Could you check a few things on this model? Use its own coordinates, in mm. A direction names the side the tool comes from. Give positions to 0.01 mm unless a question says otherwise; leave off trailing zeros. Loops run counter-clockwise (first coordinate to the right, second up) from the corner with the lowest first, then second, coordinate; pieces in that order, holes last. Notation, with made-up numbers: (-0.75, 79) - (44.25, 79) arc R14 ccw to (44.25, 84) - close; hole circle Ø7 at (-27, 71.25). An arc over 180 degrees is marked (long way). Use CSV: the item, a comma, the result in double quotes.
from build123d import *

# Parameters (mm, degrees)
SKETCH1_W           = 29
SKETCH1_H           = 15
SKETCH1_R           = 2
SKETCH1_R_2         = 1.5
BOSS_EXTRUDE1_DEPTH = 13
SKETCH3_W           = 4.75
SKETCH3_H           = 13
SKETCH3_W_2         = 18.25
CUT_EXTRUDE1_DEPTH  = 4
SKETCH5_W           = 29
SKETCH5_H           = 4
CUT_EXTRUDE2_DEPTH  = 27
SKETCH6_W           = 1.5
SKETCH6_H           = 7
CUT_EXTRUDE3_DEPTH  = 27
SKETCH7_W           = 27.5
SKETCH7_H           = 7
CUT_EXTRUDE4_DEPTH  = 7
CHAMFER1_SIZE       = 6
CHAMFER1_SIZE2      = 4
SKETCH8_W           = 6.5
SKETCH8_H           = 0.5
CUT_EXTRUDE5_DEPTH  = 9
SKETCH9_R           = 1.25
CUT_EXTRUDE6_DEPTH  = 3.25
SKETCH12_W          = 3
SKETCH12_H          = 7
CUT_EXTRUDE8_DEPTH  = 8
SKETCH13_R          = 1.5
CUT_EXTRUDE9_DEPTH  = 8
CHAMFER3_SIZE       = 1
SKETCH17_W          = 1.5
SKETCH17_H          = 7
CUT_EXTRUDE11_DEPTH = 9
CHAMFER4_SIZE       = 2
M2_TAPPED_HOLE1_D   = 1.6


with BuildPart() as part:
    # Sketch1 → Boss-Extrude1 (new body)
    with BuildSketch(Plane.XY):
        Rectangle(SKETCH1_W, SKETCH1_H)
        with Locations(Location((6.75, 0, 0), (0, 0, 180))):
            Circle(SKETCH1_R, mode=Mode.SUBTRACT)
        with Locations(Location((-4.75, 0, 0), (0, 0, 180))):
            Circle(SKETCH1_R_2, mode=Mode.SUBTRACT)
    extrude(amount=BOSS_EXTRUDE1_DEPTH)

    # Sketch3 → Cut-Extrude1 (cut)
    with BuildSketch(Plane.XZ.offset(7.5)):
        with Locations((12.125, 6.5)):
            Rectangle(SKETCH3_W, SKETCH3_H)
        with Locations((-5.375, 6.5)):
            Rectangle(SKETCH3_W_2, SKETCH3_H)
    extrude(amount=-CUT_EXTRUDE1_DEPTH, mode=Mode.SUBTRACT)

    # Sketch5 → Cut-Extrude2 (cut)
    with BuildSketch(Plane(origin=(0, 0, 0), x_dir=(-1, 0, 0), z_dir=(0, 0, -1))):
        with Locations((0, 5.5)):
            Rectangle(SKETCH5_W, SKETCH5_H)
    extrude(amount=-CUT_EXTRUDE2_DEPTH, mode=Mode.SUBTRACT)

    # Sketch6 → Cut-Extrude3 (cut)
    with BuildSketch(Plane(origin=(0, 0, 0), x_dir=(-1, 0, 0), z_dir=(0, 0, -1))):
        with Locations((13.75, 0)):
            Rectangle(SKETCH6_W, SKETCH6_H)
    extrude(amount=-CUT_EXTRUDE3_DEPTH, mode=Mode.SUBTRACT)

    # Sketch7 → Cut-Extrude4 (cut)
    with BuildSketch(Plane(origin=(0, 0, 0), x_dir=(-1, 0, 0), z_dir=(0, 0, -1))):
        with Locations((-0.75, 0)):
            Rectangle(SKETCH7_W, SKETCH7_H)
    extrude(amount=-CUT_EXTRUDE4_DEPTH, mode=Mode.SUBTRACT)

    # Chamfer1
    chamfer1_edges = [part.edges().sort_by_distance(p)[0] for p in [
        (6.75, -7.5, 13),
    ]]
    chamfer1_side = [part.faces().sort_by_distance(p)[0] for p in [
        (6.75, -7.5, 6.5),
    ]]
    chamfer(chamfer1_edges, length=CHAMFER1_SIZE, length2=CHAMFER1_SIZE2, reference=chamfer1_side[0])

    # Sketch8 → Cut-Extrude5 (cut)
    with BuildSketch(Plane(origin=(0, 0, 7), x_dir=(-1, 0, 0), z_dir=(0, 0, -1))):
        Polygon((-1.75, -3.5), (-1.75, -0.25), (3.75, -0.25), (3.75, 0.25), (-2.25, 0.25), (-2.25, -3.5), align=None)
        with Locations((-11.25, 0)):
            Rectangle(SKETCH8_W, SKETCH8_H)
    extrude(amount=-CUT_EXTRUDE5_DEPTH, mode=Mode.SUBTRACT)

    # Sketch9 → Cut-Extrude6 (cut)
    with BuildSketch(Plane.XZ.offset(3.5)):
        with Locations((12.3, 10)):
            Circle(SKETCH9_R)
        with Locations((-0.7, 10)):
            Circle(SKETCH9_R)
    extrude(amount=-CUT_EXTRUDE6_DEPTH, mode=Mode.SUBTRACT)

    # Sketch12 → Cut-Extrude8 (cut)
    with BuildSketch(Plane.XY.offset(13)):
        with Locations((-11.5, 0)):
            Rectangle(SKETCH12_W, SKETCH12_H)
    extrude(amount=-CUT_EXTRUDE8_DEPTH, mode=Mode.SUBTRACT)

    # Sketch13 → Cut-Extrude9 (cut)
    with BuildSketch(Plane.XZ.offset(7.5)):
        with Locations((6.75, 3)):
            Circle(SKETCH13_R)
    extrude(amount=-CUT_EXTRUDE9_DEPTH, mode=Mode.SUBTRACT)

    # Chamfer3
    chamfer3_edges = [part.edges().sort_by_distance(p)[0] for p in [
        (9.75, -5.5, 0),
        (3.75, -5.5, 0),
    ]]
    chamfer(chamfer3_edges, length=CHAMFER3_SIZE)

    # Sketch17 → Cut-Extrude11 (cut)
    with BuildSketch(Plane(origin=(0, 0, 7), x_dir=(-1, 0, 0), z_dir=(0, 0, -1))):
        with Locations((9.25, 0)):
            Rectangle(SKETCH17_W, SKETCH17_H)
    extrude(amount=-CUT_EXTRUDE11_DEPTH, mode=Mode.SUBTRACT)

    # Chamfer4
    chamfer4_edges = [part.edges().sort_by_distance(p)[0] for p in [
        (-8.5, -3.5, 10),
        (-8.5, 3.5, 10),
    ]]
    chamfer(chamfer4_edges, length=CHAMFER4_SIZE)

    # M2 Tapped Hole1 (through all)
    with Locations(Plane(origin=(0, 3.5, 0), x_dir=(1, 0, 0), z_dir=(0, 1, 0))):
        with Locations((-0.7, -10), (12.3, -10)):
            Hole(M2_TAPPED_HOLE1_D / 2)


solid = part.part
1) Suppose I cut it at D-D (y = -5). Please give me the cut outline in (x, z), plus the area to 3 significant figures.
Answer below:
outline,"(3.75, 1) - (4.75, 0) - (8.75, 0) - (9.75, 1) - (9.75, 10.75) - (3.75, 10.75) - close; hole circle Ø3 at (6.75, 3)"
area,"56.4 mm2"
2) I need wall thicknesses on line 1 along Z through (x, y) = (-0.7, -2.1); line 2 along Z through (x, y) = (-0.7, 1.6); line 3 along X through (y, z) = (2.75, 10). Which ranges of each line are inside material? Lowest first, please.
Answer below:
line 1,"z = 7 to 8.75, 11.25 to 13"
line 2,"z = 7 to 9.2, 10.8 to 13"
line 3,"x = -7.25 to -1.5, 0.1 to 11.5, 13.1 to 14.5"
3) We'd pull the mould along X, two halves only. Please class faces 4 (the flat face through (2.25, -2, 10)), 5 (the flat face through (7, -7.5, 5)), 6 (the flat face through (-8, -2, 10)): +X half, -X half, draft (parallel to the pull), parting line (faces both ways), or undercut.
Answer below:
face 4,"undercut"
face 5,"draft"
face 6,"-X half"
4) I'm going to push flat-ended pins straight in: P1, Ø5, axis at x = -4.75, y = 0, coming from the -Z side; P2, Ø1.5, axis at y = -2, z = 5, coming from the +X side; P3, Ø2, axis at y = -5.5, z = 7.5, coming from the -X side; P4, Ø4.5, axis at y = -5, z = 4.5, coming from the +X side. Where does each tip first touch, or does it pass through?
Answer below:
P1,"stops at z = 7"
P2,"passes through"
P3,"stops at x = 3.75"
P4,"stops at x = 9.75"
5) Suppose I cut it at A-A (x = 6.75). Please give me the cut outline in (y, z).
Answer below:
outline,"(-7.5, 0) - (-3.5, 0) - (-3.5, 1.5) - (-7.5, 1.5) - close; (-7.5, 4.5) - (-3.5, 4.5) - (-3.5, 7) - (-2, 7) - (-2, 13) - (-3.5, 13) - (-7.5, 7) - close; (2, 7) - (3.5, 7) - (3.5, 13) - (2, 13) - close"
6) Which directions (+Z, -Z, +X, -X, +Y, -Y) give clear straight access to the entire face, cutting with the end or side of a thin tool? Please do faces 1 (the flat face through (-2.4, -3.5, 10)), 2 (the cylindrical face through (-0.86, -1.9, 11.24)), 3 (the flat face through (7, -3.5, 5)).
Answer below:
face 1,"+Z, -Z, -X, -Y"
face 2,"-Y"
face 3,"-Z, +X, -X, +Y"
7) Suppose I cut it at C-C (z = 3). Please give me the cut outline in (x, y).
Answer below:
outline,"(3.75, -7.5) - (5.25, -7.5) - (5.25, -3.5) - (3.75, -3.5) - close; (8.25, -7.5) - (9.75, -7.5) - (9.75, -3.5) - (8.25, -3.5) - close"
8) Suppose I cut it at B-B (x = 12.3). Please give me the cut outline in (y, z).
Answer below:
outline,"(-3.5, 7) - (-0.25, 7) - (-0.25, 8.75) - (-3.5, 8.75) - close; (-3.5, 11.25) - (-0.25, 11.25) - (-0.25, 13) - (-3.5, 13) - close; (0.25, 7) - (3.5, 7) - (3.5, 9.2) - (0.25, 9.2) - close; (0.25, 10.8) - (3.5, 10.8) - (3.5, 13) - (0.25, 13) - close"
